```python
from build123d import *

# Parameters (mm, degrees)
SKETCH2_OUTSIDE_W   = 103.606
SKETCH2_OUTSIDE_H   = 103.606
SKETCH2_OUTSIDE_W_2 = 58
SKETCH2_OUTSIDE_H_2 = 58
CUT_EXTRUDE1_DEPTH  = 10
SKETCH3_R           = 5.5
CUT_EXTRUDE2_DEPTH  = 6.1
CUT_EXTRUDE3_REACH  = 63.703
SKETCH4_R           = 3.3
CIRPATTERN1_COUNT   = 4
FILLET1_R           = 1.5


with BuildPart() as part:
    # Sketch1 → Revolve1 (revolve)
    with BuildSketch(Plane.XY, mode=Mode.PRIVATE) as revolve1_sk:
        Polygon((0, 37), (0, 21.5), (-1, 21.5), (-1, 22.5), (-40, 22.5), (-40, 15), (0, 15), (50, 15), (50, 22.5), (11, 22.5), (11, 21.5), (10, 21.5), (10, 37), align=None)
    revolve(revolve1_sk.sketch.rotate(Axis((64, 0, 0), (-1, 0, 0)), 270), axis=Axis((64, 0, 0), (-1, 0, 0)))

    # Sketch2 outside → Cut-Extrude1 (cut)
    with BuildSketch(Plane(origin=(0, 0, 0), x_dir=(0, 0, -1), z_dir=(1, 0, 0))):
        Rectangle(SKETCH2_OUTSIDE_W, SKETCH2_OUTSIDE_H)
        Rectangle(SKETCH2_OUTSIDE_W_2, SKETCH2_OUTSIDE_H_2, mode=Mode.SUBTRACT)
    extrude(amount=CUT_EXTRUDE1_DEPTH, mode=Mode.SUBTRACT)

    # Sketch3 → Cut-Extrude2 (cut)
    with BuildSketch(Plane.ZY):
        with Locations((-21.213203436, 21.213203436)):
            Circle(SKETCH3_R)
    cut_extrude2 = extrude(amount=-CUT_EXTRUDE2_DEPTH, mode=Mode.SUBTRACT)

    # Sketch4 → Cut-Extrude3 (cut, up to next)
    with BuildSketch(Plane.ZY.offset(-6.1), mode=Mode.PRIVATE) as cut_extrude3_sk1:
        with Locations((-21.213203436, 21.213203436)):
            Circle(SKETCH4_R)
    cut_extrude3_tool1 = extrude(cut_extrude3_sk1.sketch, amount=-CUT_EXTRUDE3_REACH, mode=Mode.PRIVATE) & part.part
    cut_extrude3 = cut_extrude3_tool1.solids().sort_by_distance((6.1, 21.213203, -21.213203))[0]
    add(cut_extrude3, mode=Mode.SUBTRACT)

    # CirPattern1: Cut-Extrude2, Cut-Extrude3 ×4 about axis
    cirpattern1_axis = Axis((0, 0, 0), (1, 0, 0))
    add([cut_extrude2.rotate(cirpattern1_axis, i * 360 / CIRPATTERN1_COUNT) for i in range(1, CIRPATTERN1_COUNT)], mode=Mode.SUBTRACT)
    add([cut_extrude3.rotate(cirpattern1_axis, i * 360 / CIRPATTERN1_COUNT) for i in range(1, CIRPATTERN1_COUNT)], mode=Mode.SUBTRACT)

    # Fillet1
    fillet1_edges = [part.edges().sort_by_distance(p)[0] for p in [
        (50, 0, -22.5),
        (50, 0, -15),
        (-40, 0, -15),
        (-40, 0, -22.5),
    ]]
    fillet(fillet1_edges, radius=FILLET1_R)


solid = part.part
```
Could you check a few things on this model? Use its own coordinates, in mm. A direction names the side the tool comes from. Round coordinates to 2 decimals unless told otherwise and drop trailing zeros. Loops run counter-clockwise (first coordinate to the right, second up) from the corner with the lowest first, then second, coordinate; pieces in that order, holes last. Notation, with made-up numbers: M 69,8.5 L 96,8.5 A8 cw 96,17.5 Z; hole C -32,35.25 d9. An arc over 180 degrees is marked long. Write item = value, one per line.
1. I need wall thicknesses on probe 1 along Z at (x, y) = (-19, 8); probe 2 along X at (y, z) = (-20.5, -16); probe 3 along Y at (x, z) = (23, 12). Which ranges of each line are inside material? Lowest first, please.
Results below:
probe_1 = -21.03 to -12.69, 12.69 to 21.03
probe_2 = 6.1 to 10
probe_3 = -19.03 to -9, 9 to 19.03
2. Which directions (+Z, -Z, +X, -X, +Y, -Y) give clear straight access to the entire face, cutting with the end or side of a thin tool? Please do faces 1 (the face through (6.1, 17.6, -21.3)), 2 (the face through (8.023, -23.832, -19.205)), 3 (the face through (-0.507, 14.531, -15.846)).
Results below:
face_1 = -X
face_2 = +X, -X
face_3 = none
3. I want a section at C-C, the plane x = 3.5. Write out the boundary of the cut face in (y, z).
Results below:
outline = M -29,-22.98 A37 ccw -22.98,-29 L 22.98,-29 A37 ccw 29,-22.98 L 29,22.98 A37 ccw 22.98,29 L -22.98,29 A37 ccw -29,22.98 Z; hole C -21.21,-21.21 d11; hole C -21.21,21.21 d11; hole C 0,0 d30; hole C 21.21,-21.21 d11; hole C 21.21,21.21 d11
4. Will these pins go through, and if not, where does the flat tip stop? P1, Ø12, axis at y = 18.5, z = -24, coming from the -X side; P2, Ø10.5, axis at y = 21.21, z = -21.21, coming from the +X side; P3, Ø10, axis at x = -3.5, z = 8, coming from the -Y side; P4, Ø17.5, axis at y = 21.21, z = -21.21, coming from the +X side.
Results below:
P1 = 0
P2 = 10
P3 = -29
P4 = 49.98
5. I want a section at D-D, the plane x = -34. Write out the boundary of the cut face in (y, z).
Results below:
outline = C 0,0 d45; hole C 0,0 d30
6. Thinking about a two-plate mould opening in Z: for faces 4 (the face through (10.493, 14.531, -15.846)), 5 (the face through (-40, -11, -13)), 6 (the face through (3.007, 22.405, 15.844)), which applies, +Z half, -Z half, draft (parallel to the pull), parting line (faces both ways), or undercut?
Results below:
face_4 = parting line
face_5 = draft
face_6 = undercut
